Check sheet for the drawn part. Datum: minimum x, y, z corner. Units: mm. Give positions to 0.01 mm unless a question says otherwise; leave off trailing zeros. Loops run counter-clockwise (first coordinate to the right, second up) from the corner with the lowest first, then second, coordinate; pieces in that order, holes last. Notation, with made-up numbers: (-14, 89) - (14, 89) arc R14 ccw to (14, 102) - close; hole circle Ø7 at (-15, 20). An arc over 180 degrees is marked (long way). Use one line per item in the form item = value.
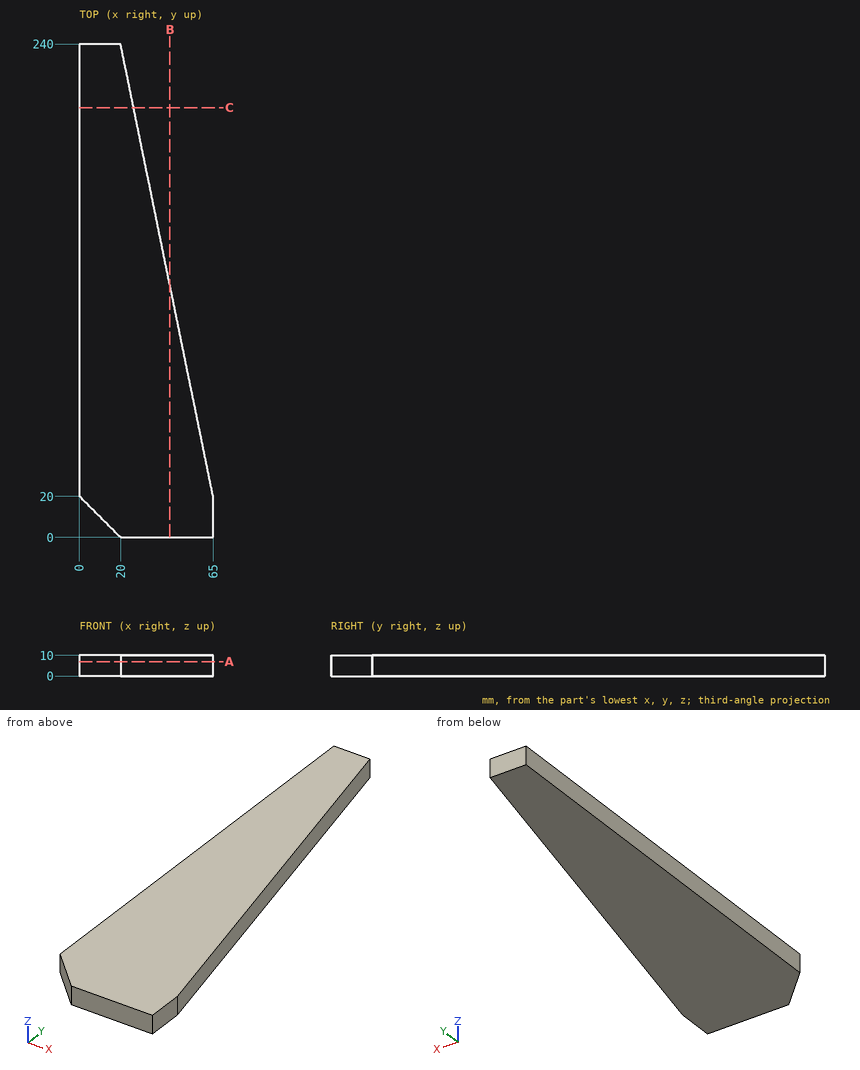
1. Section check C-C, the plane y = 209. Record the cut outline in (x, z), then the cut area to 3 significant figures.
Result set:
outline = (0, 0) - (26.34, 0) - (26.34, 10) - (0, 10) - close
area = 263 mm²
2. Scan lines: probe 1 along X at (y, z) = (99.5, 4); probe 2 along X at (y, z) = (110, 8.25); probe 3 along Y at (x, z) = (8.5, 5.25). Record each from-to range of solid material in increasing order.
Result set:
probe_1 = 0 to 48.74
probe_2 = 0 to 46.59
probe_3 = 11.5 to 240
3. Section check A-A, the plane z = 7. Record the cut outline in (x, y), then the cut area to 4 significant figures.
Result set:
outline = (0, 20) - (20, 0) - (65, 0) - (65, 20) - (20, 240) - (0, 240) - close
area = 10,450 mm²
4. Section check B-B, the plane x = 44. Record the cut outline in (y, z), then the cut area to 3 significant figures.
Result set:
outline = (0, 0) - (122.67, 0) - (122.67, 10) - (0, 10) - close
area = 1,230 mm²
5. Depth check by flat-ended pin: pin 1 Ø3 at (y, z) = (67, 8.5) entering from +X. Enter the tip coordinate at first touch or a pass-through.
Result set:
pin_1 = 55.69
